Can you work these out from the model? Positions are in its coordinate system, mm. A direction names the side the tool comes from. Give positions to 0.01 mm unless a question says otherwise; leave off trailing zeros. Loops run counter-clockwise (first coordinate to the right, second up) from the corner with the lowest first, then second, coordinate; pieces in that order, holes last. Notation, with made-up numbers: (35, 74) - (58, 74) arc R21 ccw to (58, 98) - close; hole circle Ø4 at (82, 45.25). An arc over 180 degrees is marked (long way). Write item = value, one per line.
from build123d import *

# Parameters (mm, degrees)
SKETCH1_R           = 30
BOSS_EXTRUDE1_DEPTH = 40
SKETCH2_R           = 10
CUT_EXTRUDE1_DEPTH  = 91.553851381
SKETCH3_R           = 15
CUT_EXTRUDE2_DEPTH  = 40
SKETCH4_W           = 6
SKETCH4_H           = 5.930152299
CUT_EXTRUDE3_DEPTH  = 40
SKETCH5_W           = 6.6
SKETCH5_H           = 8
CUT_EXTRUDE4_DEPTH  = 40


with BuildPart() as part:
    # Sketch1 → Boss-Extrude1 (new, symmetric)
    with BuildSketch(Plane.XY):
        Circle(SKETCH1_R)
    extrude(amount=BOSS_EXTRUDE1_DEPTH, both=True)

    # Sketch2 → Cut-Extrude1 (cut, through all)
    with BuildSketch(Plane.XY.offset(40)):
        Circle(SKETCH2_R)
    extrude(amount=-CUT_EXTRUDE1_DEPTH, mode=Mode.SUBTRACT)

    # Sketch3 → Cut-Extrude2 (cut)
    with BuildSketch(Plane(origin=(0, 0, -40), x_dir=(-1, 0, 0), z_dir=(0, 0, -1))):
        Circle(SKETCH3_R)
    extrude(amount=-CUT_EXTRUDE2_DEPTH, mode=Mode.SUBTRACT)

    # Sketch4 → Cut-Extrude3 (cut)
    with BuildSketch(Plane.XY.offset(40)):
        with Locations((0, 9.834923851)):
            Rectangle(SKETCH4_W, SKETCH4_H)
    extrude(amount=-CUT_EXTRUDE3_DEPTH, mode=Mode.SUBTRACT)

    # Sketch5 → Cut-Extrude4 (cut)
    with BuildSketch(Plane(origin=(0, 0, -40), x_dir=(-1, 0, 0), z_dir=(0, 0, -1))):
        with Locations((15, 0)):
            Rectangle(SKETCH5_W, SKETCH5_H)
    extrude(amount=-CUT_EXTRUDE4_DEPTH, mode=Mode.SUBTRACT)


solid = part.part
Q1. I need wall thicknesses on L1, parallel to Y at x = 0, z = -27; L2, parallel to Y at x = 0, z = 22; L3, parallel to Z at x = -15, y = 2. Which ranges of each line are inside material? Lowest first, please.
Output:
L1 = -30 to -15, 15 to 30
L2 = -30 to -10, 12.8 to 30
L3 = 0 to 40
Q2. Imagine slicing it at C-C, the plane z = -5.5. Write out the boundary of the cut face in (x, y).
Output:
outline = circle Ø60 at (0, 0); hole (-18.3, -4) - (-14.46, -4) arc R15 ccw (long way) to (-14.46, 4) - (-18.3, 4) - close
Q3. Which directions (+Z, -Z, +X, -X, +Y, -Y) give clear straight access to the entire face, cutting with the end or side of a thin tool? Please do faces 1 (the flat face through (6, 14, -40)), 2 (the flat face through (-18.3, 0, -20)), 3 (the flat face through (3, 11, 20)).
Output:
face_1 = -Z, +X, -X, +Y, -Y
face_2 = -Z
face_3 = +Z, -Z
Q4. We'd pull the mould along Y, two halves only. Please class faces 4 (the cylindrical face through (0, -10, 20)), 5 (the flat face through (13, 0, 40)), 6 (the cylindrical face through (-29.97, 1.32, 0.56)): released by +Y, released by -Y, zero draft, split by the parting line, or undercut.
Output:
face_4 = undercut
face_5 = zero draft
face_6 = split by the parting line
Q5. For pin 1 (10 mm diameter, centred on y = -7, z = 10, fed in from -X); pin 2 (3 mm diameter, centred on y = 2, z = -21.5, fed in from -X); pin 3 (4 mm diameter, centred on x = -17, z = -25, fed in from -Y), each with a flat end and sliding along its axis, tell me the tip position at first contact or that it passes through.
Output:
pin_1 = -29.93
pin_2 = -30
pin_3 = -25.98
Q6. Imagine slicing it at A-A, the plane x = 0. Write out the boundary of the cut face in (y, z).
Output:
outline = (-30, -40) - (-15, -40) - (-15, 0) - (-10, 0) - (-10, 40) - (-30, 40) - close; (12.8, 0) - (15, 0) - (15, -40) - (30, -40) - (30, 40) - (12.8, 40) - close
Q7. Imagine slicing it at D-D, the plane x = 14. Write out the boundary of the cut face in (y, z).
Output:
outline = (-26.53, -40) - (-5.39, -40) - (-5.39, 0) - (5.39, 0) - (5.39, -40) - (26.53, -40) - (26.53, 40) - (-26.53, 40) - close
Q8. Imagine slicing it at B-B, the plane y = 0. Write out the boundary of the cut face in (x, z).
Output:
outline = (-30, -40) - (-18.3, -40) - (-18.3, 0) - (-10, 0) - (-10, 40) - (-30, 40) - close; (10, 0) - (15, 0) - (15, -40) - (30, -40) - (30, 40) - (10, 40) - close
